Here's the drawing with two shaded views (mm, measured from the low corner). I have some questions. Give positions to 0.01 mm unless a question says otherwise; leave off trailing zeros. Loops run counter-clockwise (first coordinate to the right, second up) from the corner with the lowest first, then second, coordinate; pieces in that order, holes last. Notation, with made-up numbers: (32, 58) -> (63, 58) arc R23 cw to (63, 91) -> close; hole circle Ø6 at (-35, 49.5). An arc over 180 degrees is marked (long way). Write each question's results on one line, items separated by ' | '. Start each with the question number.
Q1. If we section it at B-B, the plane z = 17.25: List the corners of the cut face in (x, y) for me.
Q2. Will these pins go through, and if not, where does the flat tip stop? P1, Ø4, axis at x = 17.5, y = 8, coming from the -Z side; P2, Ø2, axis at x = 9, y = 9, coming from the -Z side; P3, Ø6, axis at x = 4.5, y = 2.5, coming from the +Z side.
Q3. If we section it at A-A, the plane y = 4.75: List the corners of the cut face in (x, z) for me (1 decimal).
Q4. If we section it at D-D, the plane x = 19.75: List the corners of the cut face in (y, z) for me, plus the area to 3 significant figures.
Q5. If we section it at C-C, the plane x = 5.5: List the corners of the cut face in (y, z) for me.
Q6. If I drill on line 1 along X through (y, z) = (7.25, 9.5) (1 decimal); line 2 along Z through (x, y) = (10.25, 5.25) (1 decimal); line 3 along Z through (x, y) = (9, 6.75) (1 decimal), over which ranges is the centre line in solid material (lowest first)?
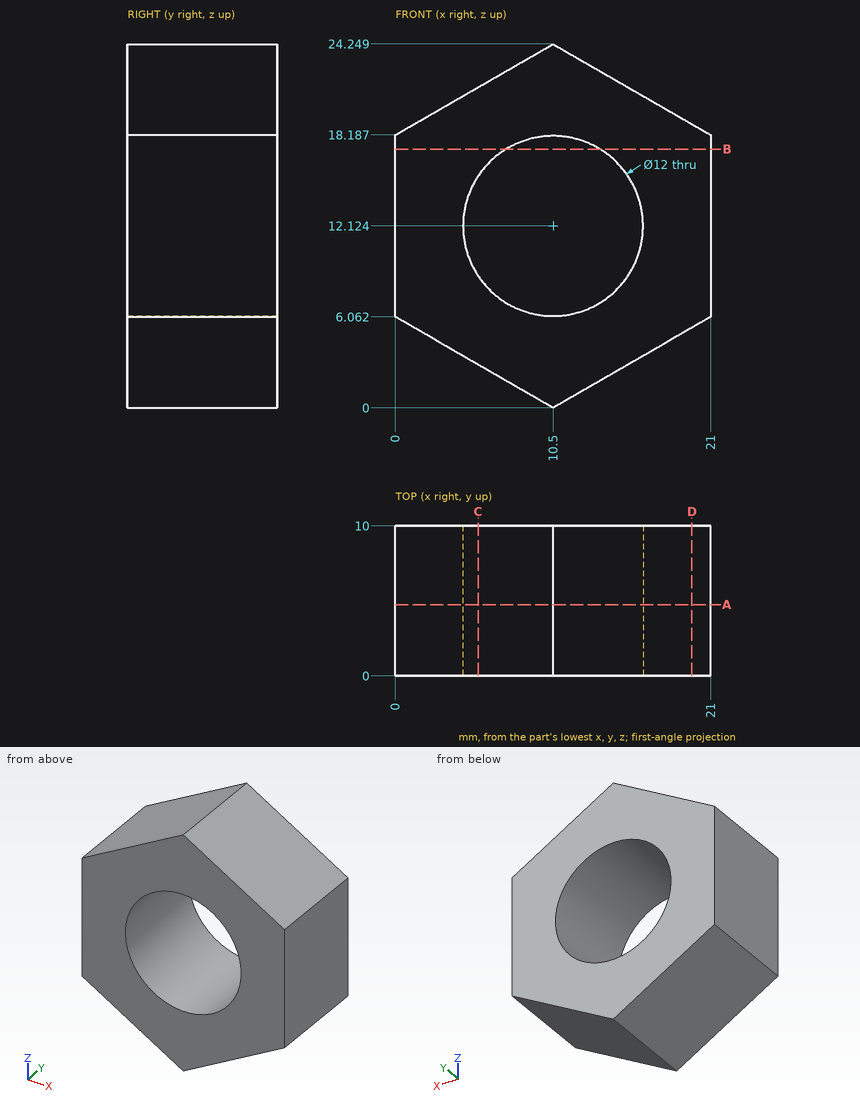
Final values:
1) outline: (0, 0) -> (7.38, 0) -> (7.38, 10) -> (0, 10) -> close; (13.62, 0) -> (21, 0) -> (21, 10) -> (13.62, 10) -> close
2) P1: stops at z = 2.89 | P2: stops at z = 0.29 | P3: stops at z = 22.52
3) outline: (0, 6.1) -> (10.5, 0) -> (21, 6.1) -> (21, 18.2) -> (10.5, 24.2) -> (0, 18.2) -> close; hole circle Ø12 at (10.5, 12.1)
4) outline: (0, 5.34) -> (10, 5.34) -> (10, 18.91) -> (0, 18.91) -> close | area: 136 mm²
5) outline: (0, 2.89) -> (10, 2.89) -> (10, 8.81) -> (0, 8.81) -> close; (0, 15.44) -> (10, 15.44) -> (10, 21.36) -> (0, 21.36) -> close
6) line 1: x = 0 to 5.1, 15.9 to 21 | line 2: z = 0.1 to 6.1, 18.1 to 24.1 | line 3: z = 0.9 to 6.3, 17.9 to 23.4
